from build123d import *

# Parameters (mm, degrees)
SKETCH_1_W             = 80
SKETCH_1_H             = 200
EXTRUDE_1_DEPTH        = 20
HOLE_WIZARD_M6_1_D     = 5
HOLE_WIZARD_M6_1_DEPTH = 20
HOLE_WIZARD_M6_1_TIP   = 1.502151548
HOLE_WIZARD_M6_2_D     = 5
HOLE_WIZARD_M6_2_DEPTH = 23
HOLE_WIZARD_M6_2_TIP   = 1.502151548


with BuildPart() as part:
    # 草图1 → 凸台-拉伸1 (new body)
    with BuildSketch(Plane(origin=(0, 0, 0), x_dir=(0, 0, -1), z_dir=(1, 0, 0))):
        Rectangle(SKETCH_1_W, SKETCH_1_H)
    extrude(amount=EXTRUDE_1_DEPTH)

    # M6 螺纹孔1
    with Locations(Plane(origin=(0, 100, 0), x_dir=(1, 0, 0), z_dir=(0, 1, 0))):
        with Locations((10, 12.5), (10, -12.5)):
            Hole(HOLE_WIZARD_M6_1_D / 2, depth=HOLE_WIZARD_M6_1_DEPTH)
            with Locations((0, 0, -(HOLE_WIZARD_M6_1_DEPTH + HOLE_WIZARD_M6_1_TIP / 2))):  # 118° drill point
                Cone(0, HOLE_WIZARD_M6_1_D / 2, HOLE_WIZARD_M6_1_TIP, mode=Mode.SUBTRACT)

    # M6 螺纹孔2
    with Locations(Plane(origin=(0, -100, 0), x_dir=(-1, 0, 0), z_dir=(0, -1, 0))):
        with Locations((-10, 20), (-10, -20)):
            Hole(HOLE_WIZARD_M6_2_D / 2, depth=HOLE_WIZARD_M6_2_DEPTH)
            with Locations((0, 0, -(HOLE_WIZARD_M6_2_DEPTH + HOLE_WIZARD_M6_2_TIP / 2))):  # 118° drill point
                Cone(0, HOLE_WIZARD_M6_2_D / 2, HOLE_WIZARD_M6_2_TIP, mode=Mode.SUBTRACT)


solid = part.part
Build history of the part. All positions in model axes, mm. A direction names the side the tool comes from. Round coordinates to 2 decimals unless told otherwise and drop trailing zeros. Answer in a Markdown table with one row per item.
Item 1: Drill centre lines: L1, parallel to Z at x = 10, y = -92; L2, parallel to Z at x = 10, y = 86.5; L3, parallel to X at y = 95, z = -12.5. Where is each one in solid material? Low to high. Write a range as [from, to].
Answers below:
| item | result |
|---|---|
| L1 | z = [-40, -22.5], [-17.5, 17.5], [22.5, 40] |
| L2 | z = [-40, -15], [-10, 10], [15, 40] |
| L3 | x = [0, 7.5], [12.5, 20] |
Item 2: Which spindle directions (+Z, -Z, +X, -X, +Y, -Y) get a long thin tool onto all of the face, cutting with end or side? Do faces 4 (the cylindrical face through (10.54, 89.86, 14.94)), 5 (the flat face through (10, -1, 40)), 6 (the cylindrical face through (9.67, -88.34, 17.52)). Say none if no direction does.
Answers below:
| item | result |
|---|---|
| face 4 | +Y |
| face 5 | +Z, +X, -X, +Y, -Y |
| face 6 | -Y |
Item 3: Pin check, flat tips, straight feed: pin 1 (3 mm diameter, centred on x = 10, z = 20, fed in from -Y); pin 2 (3 mm diameter, centred on x = 10, z = -12.5, fed in from +Y). Stop position of each tip, or through.
Answers below:
| item | result |
|---|---|
| pin 1 | stops at y = -76.4 |
| pin 2 | stops at y = 79.4 |
Item 4: Mould opens along X. For faces 1 (the flat face through (10, 100, 1)), 2 (the flat face through (20, 1, 1)), 3 (the cylindrical face through (10.54, 89.86, -10.06)) say: +X half, -X half, draft (parallel to the pull), parting line (faces both ways), or undercut.
Answers below:
| item | result |
|---|---|
| face 1 | draft |
| face 2 | +X half |
| face 3 | undercut |
